from build123d import *

# Parameters (mm, degrees)
BOSS_EXTRUDE1_DEPTH = 2.25


with BuildPart() as part:
    # Sketch1 → Boss-Extrude1 (new, symmetric)
    with BuildSketch(Plane(origin=(0, 0, 0), x_dir=(1, 0, 0), z_dir=(0, 1, 0))):
        with BuildLine():
            Line((0, 0), (25, 0))
            Line((25, 0), (25, 0.5))
            ThreePointArc((25, 0.5), (21.338834765, 9.338834765), (12.5, 13))
            Line((12.5, 13), (0, 13))
            Line((0, 13), (0, 0))
        make_face()
    extrude(amount=BOSS_EXTRUDE1_DEPTH, both=True)


solid = part.part
Could you check a few things on this model? Use its own coordinates, in mm. Coordinates: 2 decimals unless noted, no trailing zeros. Order: outer loops, then holes, each group sorted by start corner. A loop starts at its lowest first (then second) coordinate and runs counter-clockwise, first axis right, second up. Notation, with made-up numbers: (57.25, -14) -> (109.25, -14) arc R11 ccw to (109.25, -9) -> close; hole circle Ø5 at (32, 50). An arc over 180 degrees is marked (long way). One line per item, written item: value. Start each with the question number.
1) Imagine slicing it at C-C on z = -5.25. List the corners of the cut face in (x, y) for me.
2) Imagine slicing it at A-A on y = 1.2. List the corners of the cut face in (x, z) for me.
3) If I drill on L1, parallel to X at y = -0.2, z = -2.75; L2, parallel to Z at x = 12.75, y = -1.6; L3, parallel to Z at x = 19, y = 0.7, over which ranges is the centre line in solid material (lowest first)? Write a range as [from, to].
4) Imagine slicing it at B-B on x = 23.75. List the corners of the cut face in (y, z) for me.
Answer list:
1. outline: (0, -2.25) -> (24.06, -2.25) -> (24.06, 2.25) -> (0, 2.25) -> close
2. outline: (0, -13) -> (12.5, -13) arc R12.5 ccw to (25, -0.5) -> (25, 0) -> (0, 0) -> close
3. L1: x = [0, 24.8]
3. L2: z = [-13, 0]
3. L3: z = [-11.18, 0]
4. outline: (-2.25, -5.95) -> (2.25, -5.95) -> (2.25, 0) -> (-2.25, 0) -> close
